```python
from build123d import *

# Parameters (mm, degrees)
EXTRUDE_374_DEPTH      = 5.3
SKETCH_4_W             = 0.6
SKETCH_4_H             = 11.005553499
CHAMFER_1917_SIZE      = 1
FILLET_1962_R          = 0.4
PATTERN_LINEAR_1_COUNT = 16
PATTERN_LINEAR_1_PITCH = 1.25


with BuildPart() as part:
    # 草图1 → Extrude 374 (new body)
    with BuildSketch(Plane(origin=(0, 0, 0), x_dir=(0, 0, -1), z_dir=(1, 0, 0))):
        Polygon((6.5, 3.75277675), (6.5, -3.75277675), (0, -7.505553499), (-6.5, -3.75277675), (-6.5, 3.75277675), (0, 7.505553499), align=None)
    extrude(amount=EXTRUDE_374_DEPTH)

    # 草图2 → 凸台-旋转1 (revolve)
    with BuildSketch(Plane.XY, mode=Mode.PRIVATE) as revolve_1_sk:
        Polygon((0, 0), (25.3, 0), (25.3, 2.9175), (25.3, 4), (0, 4), align=None)
    revolve(revolve_1_sk.sketch.rotate(Axis((0, 0, 0), (1, 0, 0)), 90), axis=Axis((0, 0, 0), (1, 0, 0)))

    # 草图3 → 切除-旋转1 (revolve, cut)
    with BuildSketch(Plane.XY):
        Polygon((0, 6.5), (3.46730793, 12.505553499), (3.46730793, 17.505553499), (-10, 17.505553499), (-10, 6.5), align=None)
    revolve(axis=Axis((0, 0, 0), (1, 0, 0)), mode=Mode.SUBTRACT)

    # 草图5 → 切除-旋转2 (revolve, cut)
    with BuildSketch(Plane.XY):
        Polygon((5.3, 6.5), (1.83269207, 12.505553499), (1.83269207, 17.505553499), (11.83269207, 17.505553499), (11.83269207, 6.5), align=None)
    revolve(axis=Axis((0, 0, 0), (1, 0, 0)), mode=Mode.SUBTRACT)

    # 草图4 → 切除-旋转3 (revolve, cut)
    with BuildSketch(Plane.XY, mode=Mode.PRIVATE) as cut_revolve_3_sk:
        with Locations((5, 12.00277675)):
            Rectangle(SKETCH_4_W, SKETCH_4_H)
    revolve(cut_revolve_3_sk.sketch.rotate(Axis((0, 0, 0), (1, 0, 0)), 270), axis=Axis((0, 0, 0), (1, 0, 0)), mode=Mode.SUBTRACT)

    # Chamfer 1917
    chamfer_1917_edges = [part.edges().sort_by_distance(p)[0] for p in [
        (25.3, 0, -4),
    ]]
    chamfer(chamfer_1917_edges, length=CHAMFER_1917_SIZE)

    # Fillet 1962
    fillet_1962_edges = [part.edges().sort_by_distance(p)[0] for p in [
        (5.3, 0, -4),
    ]]
    fillet(fillet_1962_edges, radius=FILLET_1962_R)

    # 草图6 → 切除-旋转4 (revolve, cut)
    with BuildSketch(Plane.XY):
        Polygon((6.324981666, -2.9175), (5.7, -4), (5.7, -5), (6.949963333, -5), (6.949963333, -4), align=None)
    cut_revolve_4 = revolve(axis=Axis((-3.175, 0, 0), (1, 0, 0)), mode=Mode.SUBTRACT)

    # 阵列(线性)1: 切除-旋转4 ×16
    with Locations(*[(i * PATTERN_LINEAR_1_PITCH, 0, 0) for i in range(1, PATTERN_LINEAR_1_COUNT)]):
        add(cut_revolve_4, mode=Mode.SUBTRACT)


solid = part.part
```
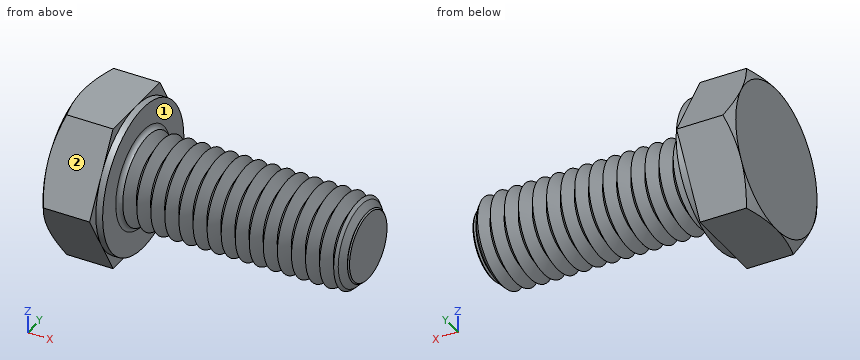
Geometry: final body of the model. Coordinates: model frame, mm. Face numbers are marked on the shaded views. A direction names the side the tool comes from. Round coordinates to 2 decimals unless told otherwise and drop trailing zeros. Write each loop counter-clockwise with the first axis right and the second up, starting at its lowest first coordinate (ties: lowest second). Pieces come first, ordered by that corner, then holes. Notation, with made-up numbers: (55, -34) -> (73, -34) arc R8 ccw to (73, -20) -> close; hole circle Ø8 at (89.5, -34.5). An arc over 180 degrees is marked (long way). Return JSON: item names as keys, results as strings.
Q1. Ray query, line 1 (X direction, y = 3, z = 3.5); line 2 (Z direction, x = 18, y = 1.5); line 3 (Y direction, x = 24.25, z = -1). Return the intervals inside material, ascending.
From the geometry:
{"line 1": "0 to 5.3", "line 2": "-3.33 to 3.33", "line 3": "-3.51 to 3.51"}
Q2. Section A-A on x = 9.75. Return the cut outline in (y, z).
From the geometry:
{"outline": "circle Ø6.96 at (0, 0)"}
Q3. First-contact query: pin 1 Ø2.5 at (y, z) = (-1.5, 4.5) entering from +X; pin 2 Ø2 at (y, z) = (4, -2) entering from +X; pin 3 Ø1.6 at (y, z) = (2, 4.5) entering from +X. Flat tips, straight axial feed; report the tip coordinate or a pass-through.
From the geometry:
{"pin 1": "x = 24.74", "pin 2": "x = 24.75", "pin 3": "x = 5.41"}
Q4. Set-up query: the marked faces 1 and 2. Return all of +Z, -Z, +X, -X, +Y, -Y with unobstructed straight access to the full face (end or side cutting, diameter ignored); none if empty.
From the geometry:
{"face 1": "+X", "face 2": "+Z, +X, -X, -Y"}
